Check sheet for the modelled part. Datum: model origin and axes. Units: mm. Give positions to 0.01 mm unless a question says otherwise; leave off trailing zeros. Order: outer loops, then holes, each group sorted by start corner. A loop starts at its lowest first (then second) coordinate and runs counter-clockwise, first axis right, second up.
Item 1: Sectioned sample at C-C on y = 5.75. Record the boundary of the cut face in (x, z), and give its area (3 significant figures).
Item 2: Release check for a two-part mould opening along Z. For faces 1 (the cylindrical face through (48.49, 3.13, 1.2)), 2 (the flat face through (26, 3, 5.08)), 3 (the cylindrical face through (0.782, 3.131, 2.483)), 4 (the flat face through (25, 3, -5.08)) record: released by +Z, released by -Z, zero draft, split by the parting line, or undercut.
Item 3: Sectioned sample at D-D on x = 49.5. Record the boundary of the cut face in (y, z).
Item 4: Sectioned sample at A-A on x = 25.4. Record the boundary of the cut face in (y, z).
Item 5: Material ranges on line 1 along X through (y, z) = (5, 0); line 2 along X through (y, z) = (2.75, 1.75); line 3 along Z through (x, y) = (1, 5.25), recorded low to high.
Item 6: Sectioned sample at B-B on z = 0. Record the boundary of the cut face in (x, y), and give its area (3 significant figures).
from build123d import *

# Parameters (mm, degrees)
SKETCH1_R           = 2.9
BOSS_EXTRUDE1_DEPTH = 6.35
BOSS_EXTRUDE2_START = -6.35
SKETCH2_R           = 2.9
SKETCH2_R_2         = 2.6035
BOSS_EXTRUDE2_DEPTH = 6.35
SKETCH2_2_R         = 2.6035
CUT_EXTRUDE1_DEPTH  = 57.468604552


with BuildPart() as part:
    # Sketch1 → Boss-Extrude1 (new body)
    with BuildSketch(Plane(origin=(0, 0, 0), x_dir=(1, 0, 0), z_dir=(0, 1, 0))):
        with BuildLine():
            Line((0, 5.08), (50.8, 5.08))
            ThreePointArc((50.8, 5.08), (55.88, 0), (50.8, -5.08))
            Line((50.8, -5.08), (0, -5.08))
            ThreePointArc((0, -5.08), (-5.08, 0), (0, 5.08))
        make_face()
        with Locations(Location((0, 0, 0), (0, 0, 270))):
            Circle(SKETCH1_R, mode=Mode.SUBTRACT)
        with Locations(Location((50.8, 0, 0), (0, 0, 270))):
            Circle(SKETCH1_R, mode=Mode.SUBTRACT)
    extrude(amount=BOSS_EXTRUDE1_DEPTH)

    # Sketch2 → Boss-Extrude2 (add)
    # profile 1 of 3: a face of its own
    with BuildSketch(Plane(origin=(0, 6.35, 0), x_dir=(1, 0, 0), z_dir=(0, 1, 0)).offset(BOSS_EXTRUDE2_START)):
        Circle(SKETCH2_R)
        with Locations(Location((0, 0, 0), (0, 0, 270))):
            Circle(SKETCH2_R_2, mode=Mode.SUBTRACT)
    # profile 2 of 3: a face of its own
    with BuildSketch(Plane(origin=(0, 6.35, 0), x_dir=(1, 0, 0), z_dir=(0, 1, 0)).offset(BOSS_EXTRUDE2_START)):
        with Locations((50.8, 0)):
            Circle(SKETCH2_R)
        with Locations(Location((50.8, 0, 0), (0, 0, 270))):
            Circle(SKETCH2_R_2, mode=Mode.SUBTRACT)
    # profile 3 of 3: a face of its own
    with BuildSketch(Plane(origin=(0, 6.35, 0), x_dir=(1, 0, 0), z_dir=(0, 1, 0)).offset(BOSS_EXTRUDE2_START)):
        with Locations((25.4, 0)):
            Circle(SKETCH2_R_2)
    extrude(amount=BOSS_EXTRUDE2_DEPTH)

    # Sketch2<2> → Cut-Extrude1 (cut, through all)
    with BuildSketch(Plane(origin=(0, 6.35, 0), x_dir=(1, 0, 0), z_dir=(0, 1, 0))):
        with Locations(Location((25.4, 0, 0), (0, 0, 270))):
            Circle(SKETCH2_2_R)
    extrude(amount=-CUT_EXTRUDE1_DEPTH, mode=Mode.SUBTRACT)


solid = part.part
Report:
1. outline: (0, -5.08) - (50.8, -5.08) arc R5.08 ccw to (50.8, 5.08) - (0, 5.08) arc R5.08 ccw to start; hole circle Ø5.21 at (0, 0); hole circle Ø5.21 at (25.4, 0); hole circle Ø5.21 at (50.8, 0)
1. area: 533 mm2
2. face 1: undercut
2. face 2: released by +Z
2. face 3: undercut
2. face 4: released by -Z
3. outline: (0, -5.08) - (6.35, -5.08) - (6.35, -2.26) - (0, -2.26) - close; (0, 2.26) - (6.35, 2.26) - (6.35, 5.08) - (0, 5.08) - close
4. outline: (0, -5.08) - (6.35, -5.08) - (6.35, -2.6) - (0, -2.6) - close; (0, 2.6) - (6.35, 2.6) - (6.35, 5.08) - (0, 5.08) - close
5. line 1: x = -5.08 to -2.6, 2.6 to 22.8, 28 to 48.2, 53.4 to 55.88
5. line 2: x = -4.77 to -1.93, 1.93 to 23.47, 27.33 to 48.87, 52.73 to 55.57
5. line 3: z = -5.08 to -2.4, 2.4 to 5.08
6. outline: (-5.08, 0) - (-2.6, 0) - (-2.6, 6.35) - (-5.08, 6.35) - close; (2.6, 0) - (22.8, 0) - (22.8, 6.35) - (2.6, 6.35) - close; (28, 0) - (48.2, 0) - (48.2, 6.35) - (28, 6.35) - close; (53.4, 0) - (55.88, 0) - (55.88, 6.35) - (53.4, 6.35) - close
6. area: 288 mm2
